from build123d import *

# Parameters (mm, degrees)
EXTRUDE1_DEPTH         = 1232
SKETCH2_W              = 32
SKETCH2_H              = 32
CUT_EXTRUDE1_DEPTH     = 1236.242486316
SKETCH3_W              = 32
SKETCH3_H              = 4
CUT_EXTRUDE2_DEPTH     = 1200
CUT_EXTRUDE3_DEPTH     = 10
LPATTERN1_COUNT        = 5
LPATTERN1_PITCH        = 40
LPATTERN2_COUNT        = 2
LPATTERN2_PITCH        = 350
LPATTERN2_COPY_1_DEPTH = 10
LPATTERN2_COPY_2_DEPTH = 10
LPATTERN2_COPY_3_DEPTH = 10
LPATTERN2_COPY_4_DEPTH = 10


with BuildPart() as part:
    # Sketch1 → Extrude1 (new body)
    with BuildSketch(Plane.XY):
        Polygon((0, 0), (-40, 0), (-40, 80), (0, 80), (0, 76), (-32, 76), (-32, 4), (0, 4), align=None)
    extrude(amount=EXTRUDE1_DEPTH)

    # Sketch2 → Cut-Extrude1 (cut, through all)
    with BuildSketch(Plane(origin=(0, 80, 0), x_dir=(1, 0, 0), z_dir=(0, 1, 0))):
        with Locations((-16, -16)):
            Rectangle(SKETCH2_W, SKETCH2_H)
        with Locations((-16, -1216)):
            Rectangle(SKETCH2_W, SKETCH2_H)
    extrude(amount=-CUT_EXTRUDE1_DEPTH, mode=Mode.SUBTRACT)

    # Sketch3 → Cut-Extrude2 (cut)
    with BuildSketch(Plane(origin=(-32, 0, 0), x_dir=(0, 0, -1), z_dir=(1, 0, 0))):
        with Locations((-1216, 78)):
            Rectangle(SKETCH3_W, SKETCH3_H)
        with Locations((-1216, 2)):
            Rectangle(SKETCH3_W, SKETCH3_H)
        with Locations((-16, 78)):
            Rectangle(SKETCH3_W, SKETCH3_H)
        with Locations((-16, 2)):
            Rectangle(SKETCH3_W, SKETCH3_H)
    extrude(amount=-CUT_EXTRUDE2_DEPTH, mode=Mode.SUBTRACT)

    # Sketch4 → Cut-Extrude3 (cut)
    with BuildSketch(Plane(origin=(0, 80, 0), x_dir=(1, 0, 0), z_dir=(0, 1, 0))):
        with BuildLine():
            Line((-24.5, -937.25), (-24.5, -962.75))
            ThreePointArc((-24.5, -962.75), (-20, -967.25), (-15.5, -962.75))
            Line((-15.5, -962.75), (-15.5, -937.25))
            ThreePointArc((-15.5, -937.25), (-20, -932.75), (-24.5, -937.25))
        make_face()
    cut_extrude3 = extrude(amount=-CUT_EXTRUDE3_DEPTH, mode=Mode.SUBTRACT)

    # LPattern1: Cut-Extrude3 ×5
    with Locations(*[(0, 0, -i * LPATTERN1_PITCH) for i in range(1, LPATTERN1_COUNT)]):
        add(cut_extrude3, mode=Mode.SUBTRACT)

    # LPattern2: Cut-Extrude3 ×2
    with Locations(*[(0, 0, -i * LPATTERN2_PITCH) for i in range(1, LPATTERN2_COUNT)]):
        add(cut_extrude3, mode=Mode.SUBTRACT)

    # LPattern2 copy 1 sketch → LPattern2 copy 1 (cut)
    with BuildSketch(Plane(origin=(0, 80, -390), x_dir=(1, 0, 0), z_dir=(0, 1, 0))):
        with BuildLine():
            Line((-24.5, -937.25), (-24.5, -962.75))
            ThreePointArc((-24.5, -962.75), (-20, -967.25), (-15.5, -962.75))
            Line((-15.5, -962.75), (-15.5, -937.25))
            ThreePointArc((-15.5, -937.25), (-20, -932.75), (-24.5, -937.25))
        make_face()
    extrude(amount=-LPATTERN2_COPY_1_DEPTH, mode=Mode.SUBTRACT)

    # LPattern2 copy 2 sketch → LPattern2 copy 2 (cut)
    with BuildSketch(Plane(origin=(0, 80, -430), x_dir=(1, 0, 0), z_dir=(0, 1, 0))):
        with BuildLine():
            Line((-24.5, -937.25), (-24.5, -962.75))
            ThreePointArc((-24.5, -962.75), (-20, -967.25), (-15.5, -962.75))
            Line((-15.5, -962.75), (-15.5, -937.25))
            ThreePointArc((-15.5, -937.25), (-20, -932.75), (-24.5, -937.25))
        make_face()
    extrude(amount=-LPATTERN2_COPY_2_DEPTH, mode=Mode.SUBTRACT)

    # LPattern2 copy 3 sketch → LPattern2 copy 3 (cut)
    with BuildSketch(Plane(origin=(0, 80, -470), x_dir=(1, 0, 0), z_dir=(0, 1, 0))):
        with BuildLine():
            Line((-24.5, -937.25), (-24.5, -962.75))
            ThreePointArc((-24.5, -962.75), (-20, -967.25), (-15.5, -962.75))
            Line((-15.5, -962.75), (-15.5, -937.25))
            ThreePointArc((-15.5, -937.25), (-20, -932.75), (-24.5, -937.25))
        make_face()
    extrude(amount=-LPATTERN2_COPY_3_DEPTH, mode=Mode.SUBTRACT)

    # LPattern2 copy 4 sketch → LPattern2 copy 4 (cut)
    with BuildSketch(Plane(origin=(0, 80, -510), x_dir=(1, 0, 0), z_dir=(0, 1, 0))):
        with BuildLine():
            Line((-24.5, -937.25), (-24.5, -962.75))
            ThreePointArc((-24.5, -962.75), (-20, -967.25), (-15.5, -962.75))
            Line((-15.5, -962.75), (-15.5, -937.25))
            ThreePointArc((-15.5, -937.25), (-20, -932.75), (-24.5, -937.25))
        make_face()
    extrude(amount=-LPATTERN2_COPY_4_DEPTH, mode=Mode.SUBTRACT)


solid = part.part
Geometry check sheet. Reference: the model listing, model coordinates, mm. A direction names the side the tool comes from. Round coordinates to 2 decimals unless told otherwise and drop trailing zeros. Loops run counter-clockwise (first coordinate to the right, second up) from the corner with the lowest first, then second, coordinate; pieces in that order, holes last. Notation, with made-up numbers: (-20, 87) -> (30, 87) arc R28 ccw to (30, 113) -> close; hole circle Ø2 at (81.5, 20). An arc over 180 degrees is marked (long way). Answer as a JSON object with one key per item and string values. Group by question number.
Item 1: Release check for a two-part mould opening along Y. For faces 1 (the face through (-16, 4, 608)), 2 (the face through (-12, 76, 608)), 3 (the face through (-25, 80, 608)), 4 (the face through (-40, 39, 607)) record: pulls with the +Y half, pulls with the -Y half, needs draft (parallel to the pull), parting line crosses it, or undercut.
Item 2: Cross-section at C-C, the plane y = 65. Record the cut outline in (x, z).
Item 3: Cross-section at B-B, the plane z = 261.5. Record the cut outline in (x, y), plus the area to 3 significant figures.
Item 4: Thickness scan on line 1 along Y through (x, z) = (-13, 958.5); line 2 along X through (y, z) = (49, 1148). Record the ranges inside material, lowest first.
Item 5: Depth check by flat-ended pin: pin 1 Ø1.2 at (y, z) = (77, 476.5) entering from +X; pin 2 Ø8 at (y, z) = (47, 228.5) entering from +X; pin 3 Ø9 at (x, z) = (-35, 15) entering from +Y; pin 4 Ø3 at (x, y) = (-18, 2) entering from +Z. Enter the tip coordinate at first touch or a pass-through.
Item 6: Cross-section at A-A, the plane z = 517.5. Record the cut outline in (x, y).
Item 7: Set-up check for faces 5 (the face through (-32, 41, 625)), 6 (the face through (-20, 0, 608)): record each of +Z, -Z, +X, -X, +Y, -Y from which the full face is reachable in a straight line by a thin tool's end or side.
Determined:
{
 "1": {"face 1": "undercut", "face 2": "undercut", "face 3": "pulls with the +Y half", "face 4": "needs draft"},
 "2": {"outline": "(-40, 0) -> (-32, 0) -> (-32, 1232) -> (-40, 1232) -> close"},
 "3": {"outline": "(-40, 0) -> (0, 0) -> (0, 4) -> (-32, 4) -> (-32, 76) -> (0, 76) -> (0, 80) -> (-40, 80) -> close", "area": "896 mm²"},
 "4": {"line 1": "y = 0 to 4, 76 to 80", "line 2": "x = -40 to -32"},
 "5": {"pin 1": "stops at x = 0", "pin 2": "stops at x = -32", "pin 3": "stops at y = 76", "pin 4": "stops at z = 1200"},
 "6": {"outline": "(-40, 0) -> (0, 0) -> (0, 4) -> (-32, 4) -> (-32, 76) -> (-24.5, 76) -> (-24.5, 80) -> (-40, 80) -> close; (-15.5, 76) -> (0, 76) -> (0, 80) -> (-15.5, 80) -> close"},
 "7": {"face 5": "+Z, -Z, +X", "face 6": "+Z, -Z, +X, -X, -Y"}
}
